```python
from build123d import *

# Parameters (mm, degrees)
SKETCH_1_W          = 60
SKETCH_1_H          = 437.5
EXTRUDE_1_DEPTH     = 3
CHAMFER_1_SIZE      = 10
SKETCH_2_R          = 5
CUT_EXTRUDE_1_DEPTH = 10


with BuildPart() as part:
    # 草图1 → 凸台-拉伸1 (new body)
    with BuildSketch(Plane.XY):
        with Locations((0, -18.75)):
            Rectangle(SKETCH_1_W, SKETCH_1_H)
    extrude(amount=EXTRUDE_1_DEPTH)

    # 倒角1
    chamfer_1_edges = [part.edges().sort_by_distance(p)[0] for p in [
        (30, -237.5, 1.5),
        (-30, -237.5, 1.5),
        (-30, 200, 1.5),
        (30, 200, 1.5),
    ]]
    chamfer(chamfer_1_edges, length=CHAMFER_1_SIZE)

    # 草图2 → 切除-拉伸1 (cut)
    with BuildSketch(Plane.XY.offset(3)):
        with Locations((0, 99)):
            Circle(SKETCH_2_R)
        with Locations((0, -117.75)):
            Circle(SKETCH_2_R)
        with BuildLine():
            Line((6.5, 50.5), (6.5, 45.5))
            ThreePointArc((6.5, 45.5), (0, 39), (-6.5, 45.5))
            Line((-6.5, 45.5), (-6.5, 50.5))
            ThreePointArc((-6.5, 50.5), (0, 57), (6.5, 50.5))
        make_face()
        with BuildLine():
            Line((6.5, -45.5), (6.5, -50.5))
            ThreePointArc((6.5, -50.5), (0, -57), (-6.5, -50.5))
            Line((-6.5, -50.5), (-6.5, -45.5))
            ThreePointArc((-6.5, -45.5), (0, -39), (6.5, -45.5))
        make_face()
    extrude(amount=-CUT_EXTRUDE_1_DEPTH, mode=Mode.SUBTRACT)


solid = part.part
```
Can you work these out from the model? Positions are in its coordinate system, mm. Give positions to 0.01 mm unless a question says otherwise; leave off trailing zeros. Write each loop counter-clockwise with the first axis right and the second up, starting at its lowest first coordinate (ties: lowest second). Pieces come first, ordered by that corner, then holes. Notation, with made-up numbers: (48, 17) - (105, 17) arc R22 ccw to (105, 24) - close; hole circle Ø4 at (26, -6). An arc over 180 degrees is marked (long way). Write item = value, one per line. Start each with the question number.
1. Please list where these lines run through material, in increasing order: line 1 (Y direction, x = 0, z = 0.85); line 2 (Y direction, x = 2, z = 2.65); line 3 (Y direction, x = -21.5, z = 1.15).
2. Thinking about a two-plate mould opening in Y: for faces 1 (the face through (2.688, -113.534, 1.521)), 2 (the face through (25.1, -232.4, 1.5)), 3 (the face through (0, -16, 0)), 4 (the face through (-1.08, 94.12, 1.52)), which applies, released by +Y, released by -Y, zero draft, split by the parting line, or undercut?
3. Imagine slicing it at A-A (y = -117.75). Please give me the cut outline in (x, z), and give its area (3 significant figures).
4. Imagine slicing it at B-B (z = 1.8). Please give me the cut outline in (x, y).
Worked answers:
q1.line_1 = -237.5 to -122.75, -112.75 to -57, -39 to 39, 57 to 94, 104 to 200
q1.line_2 = -237.5 to -122.33, -113.17 to -56.68, -39.32 to 39.32, 56.68 to 94.42, 103.58 to 200
q1.line_3 = -236 to 198.5
q2.face_1 = undercut
q2.face_2 = released by -Y
q2.face_3 = zero draft
q2.face_4 = undercut
q3.outline = (-30, 0) - (-5, 0) - (-5, 3) - (-30, 3) - close; (5, 0) - (30, 0) - (30, 3) - (5, 3) - close
q3.area = 150 mm2
q4.outline = (-30, -227.5) - (-20, -237.5) - (20, -237.5) - (30, -227.5) - (30, 190) - (20, 200) - (-20, 200) - (-30, 190) - close; hole (-6.5, -50.5) arc R6.5 ccw to (6.5, -50.5) - (6.5, -45.5) arc R6.5 ccw to (-6.5, -45.5) - close; hole (-6.5, 45.5) arc R6.5 ccw to (6.5, 45.5) - (6.5, 50.5) arc R6.5 ccw to (-6.5, 50.5) - close; hole circle Ø10 at (0, -117.75); hole circle Ø10 at (0, 99)
